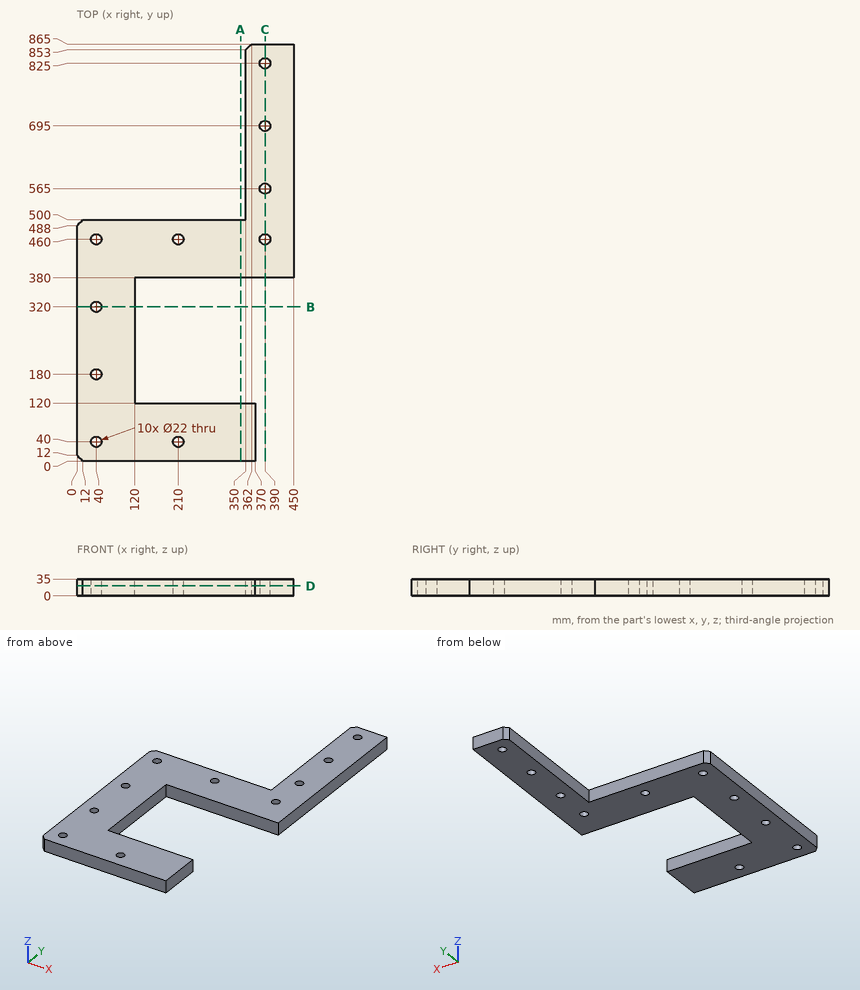
Input: dimensioned drawing with shaded views. Units: mm. Origin: part minimum x, y, z. Coordinates: 2 decimals unless noted, no trailing zeros. Loops run counter-clockwise (first coordinate to the right, second up) from the corner with the lowest first, then second, coordinate; pieces in that order, holes last. Notation, with made-up numbers: M -5.75,-0.75 L 47.25,-0.75 A28 ccw 47.25,36.25 Z; hole C 79.5,-26 d2. An arc over 180 degrees is marked long. One line per item, written item: value. Start each with the question number.
1) Pin query (flat end, axial travel): P1, Ø10.5, axis at y = 599, z = 14.5, coming from the -X side; P2, Ø17.5, axis at x = 306, z = 21.5, coming from the +Y side; P3, Ø17.5, axis at y = 192.5, z = 18, coming from the +X side; P4, Ø17.5, axis at x = 390, y = 695, coming from the -Z side. Return the tip coordinate at first contact, or that it passes through.
2) Cut plane C-C (x = 390). Return loops of the section in (y, z), then the cut area to 3 significant figures.
3) Cut plane B-B (y = 320). Return loops of the section in (x, z), then the cut area to 3 significant figures.
4) Cut plane A-A (x = 339.5). Return loops of the section in (y, z), then the cut area to 3 significant figures.
5) Material intervals for L1, parallel to Y at x = 390, z = 26; L2, parallel to Y at x = 367, z = 20; L3, parallel to Y at x = 251, z = 8, sorted ascending. Write a range as from..to.
6) Cut plane D-D (z = 21). Count the separate pieces of the cut face and the enclosed holes in it, then the cut area to 3 significant figures.
Evaluation:
1. P1: x = 350
1. P2: y = 500
1. P3: x = 120
1. P4: through
2. outline: M 380,0 L 449,0 L 449,35 L 380,35 Z; M 471,0 L 554,0 L 554,35 L 471,35 Z; M 576,0 L 684,0 L 684,35 L 576,35 Z; M 706,0 L 814,0 L 814,35 L 706,35 Z; M 836,0 L 865,0 L 865,35 L 836,35 Z
2. area: 13,900 mm^2
3. outline: M 0,0 L 29,0 L 29,35 L 0,35 Z; M 51,0 L 120,0 L 120,35 L 51,35 Z
3. area: 3,430 mm^2
4. outline: M 0,0 L 120,0 L 120,35 L 0,35 Z; M 380,0 L 500,0 L 500,35 L 380,35 Z
4. area: 8,400 mm^2
5. L1: 380..449, 471..554, 576..684, 706..814, 836..865
5. L2: 0..120, 380..865
5. L3: 0..120, 380..500
6. separate pieces: 1
6. enclosed holes: 10
6. area: 162,000 mm^2
